Design review of the part built by this model. Coordinates are the model's own, in mm. Round coordinates to 2 decimals unless told otherwise and drop trailing zeros. Order: outer loops, then holes, each group sorted by start corner. A loop starts at its lowest first (then second) coordinate and runs counter-clockwise, first axis right, second up. Notation, with made-up numbers: (20, 38.5) - (37, 38.5) arc R20 ccw to (37, 76.5) - close; hole circle Ø6 at (60.25, 41.25). An arc over 180 degrees is marked (long way). Write item = value, one per line.
from build123d import *

# Parameters (mm, degrees)
SKETCH_1_W                    = 615
SKETCH_1_H                    = 845
EXTRUDE_1_DEPTH               = 20
SKETCH_2_W                    = 615
SKETCH_2_H                    = 30
CUT_EXTRUDE_1_DEPTH           = 13
SKETCH_3_W                    = 30
SKETCH_3_H                    = 785
CUT_EXTRUDE_2_DEPTH           = 13
HOLE_WIZARD_M4_1_D            = 4
PATTERN_LINEAR_3_COUNT        = 8
PATTERN_LINEAR_3_PITCH        = 101
PATTERN_LINEAR_4_COUNT        = 6
PATTERN_LINEAR_4_PITCH        = 97
SKETCH_15_W                   = 617
SKETCH_15_H                   = 847
SKETCH_15_W_2                 = 615
SKETCH_15_H_2                 = 845
EXTRUDE_5_DEPTH               = 7
SKETCH_17_R                   = 2.5
CUT_EXTRUDE_3_DEPTH           = 20
HOLE_WIZARD_M12_2_D           = 13.5
HOLE_WIZARD_M12_2_CBORE_D     = 19
HOLE_WIZARD_M12_2_CBORE_DEPTH = 12.5
PATTERN_LINEAR_7_COUNT        = 2
PATTERN_LINEAR_7_PITCH        = 680


with BuildPart() as part:
    # 草图1 → 拉伸1 (new body)
    with BuildSketch(Plane(origin=(0, 0, 0), x_dir=(1, 0, 0), z_dir=(0, 1, 0))):
        with Locations((307.5, 422.5)):
            Rectangle(SKETCH_1_W, SKETCH_1_H)
    extrude(amount=EXTRUDE_1_DEPTH)

    # 草图2 → 切除-拉伸1 (cut)
    with BuildSketch(Plane(origin=(0, 20, 0), x_dir=(-1, 0, 0), z_dir=(0, 1, 0))):
        with Locations((-307.5, -830)):
            Rectangle(SKETCH_2_W, SKETCH_2_H)
        with Locations((-307.5, -15)):
            Rectangle(SKETCH_2_W, SKETCH_2_H)
    extrude(amount=-CUT_EXTRUDE_1_DEPTH, mode=Mode.SUBTRACT)

    # 草图3 → 切除-拉伸2 (cut)
    with BuildSketch(Plane(origin=(0, 20, 0), x_dir=(-1, 0, 0), z_dir=(0, 1, 0))):
        with Locations((-600, -422.5)):
            Rectangle(SKETCH_3_W, SKETCH_3_H)
        with Locations((-15, -422.5)):
            Rectangle(SKETCH_3_W, SKETCH_3_H)
    extrude(amount=-CUT_EXTRUDE_2_DEPTH, mode=Mode.SUBTRACT)

    # M4 螺纹孔1 (through all)
    with Locations(Plane(origin=(598.5, 7, -826.5), x_dir=(0, 0, 1), z_dir=(0, 1, 0))):
        with Locations((0, 0), (0, -582), (808, -582), (808, 0)):
            hole_wizard_m4_1 = Hole(HOLE_WIZARD_M4_1_D / 2)

    # 阵列(线性)3: M4 螺纹孔1 ×8
    with Locations(*[(0, 0, i * PATTERN_LINEAR_3_PITCH) for i in range(1, PATTERN_LINEAR_3_COUNT)]):
        add(hole_wizard_m4_1, mode=Mode.SUBTRACT)

    # 阵列(线性)4: M4 螺纹孔1 ×6
    with Locations(*[(-i * PATTERN_LINEAR_4_PITCH, 0, 0) for i in range(1, PATTERN_LINEAR_4_COUNT)]):
        add(hole_wizard_m4_1, mode=Mode.SUBTRACT)

    # 草图15 → 凸台-拉伸5 (add)
    with BuildSketch(Plane(origin=(0, 7, 0), x_dir=(1, 0, 0), z_dir=(0, 1, 0))):
        with Locations((307.5, 422.5)):
            Rectangle(SKETCH_15_W, SKETCH_15_H)
        with Locations((307.5, 422.5)):
            Rectangle(SKETCH_15_W_2, SKETCH_15_H_2, mode=Mode.SUBTRACT)
    extrude(amount=-EXTRUDE_5_DEPTH)

    # 草图17 → 切除-拉伸3 (cut)
    with BuildSketch(Plane(origin=(0, 20, 0), x_dir=(1, 0, 0), z_dir=(0, 1, 0))):
        with Locations(Location((77.5, 82.5, 0), (0, 0, 270))):
            Circle(SKETCH_17_R)
        with Locations(Location((537.5, 82.5, 0), (0, 0, 270))):
            Circle(SKETCH_17_R)
    extrude(amount=-CUT_EXTRUDE_3_DEPTH, mode=Mode.SUBTRACT)

    # M12 六角头螺栓的柱形沉头孔2 (through all)
    with Locations(Plane(origin=(0, 20, 0), x_dir=(-1, 0, 0), z_dir=(0, 1, 0))):
        with Locations((-77.5, -82.5), (-537.5, -82.5)):
            hole_wizard_m12_2 = CounterBoreHole(HOLE_WIZARD_M12_2_D / 2, HOLE_WIZARD_M12_2_CBORE_D / 2, HOLE_WIZARD_M12_2_CBORE_DEPTH)

    # 阵列(线性)7: M12 六角头螺栓的柱形沉头孔2 ×2
    with Locations(*[(0, 0, -i * PATTERN_LINEAR_7_PITCH) for i in range(1, PATTERN_LINEAR_7_COUNT)]):
        add(hole_wizard_m12_2, mode=Mode.SUBTRACT)


solid = part.part
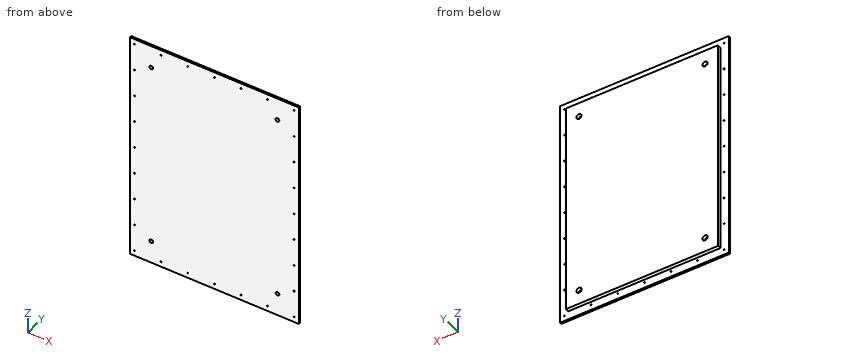
1) To check wall thickness, follow L1, parallel to Z at x = 404.5, y = 5.25; L2, parallel to X at y = 5.75, z = -762.5; L3, parallel to X at y = 17.5, z = -762.5. State the ranges of each line that lie inside material, in increasing order. Write a range as from..to.
Findings:
L1 = -846..-828.5, -824.5..-20.5, -16.5..1
L2 = -1..70.75, 84.25..530.75, 544.25..616
L3 = 30..68, 87..528, 547..585
2) Clearance check with flat-ended pins moving along their axes: pin 1 Ø10.5 at (y, z) = (16.5, -566.5) entering from +X; pin 2 Ø4.5 at (x, z) = (16.5, -321.5) entering from +Y; pin 3 Ø1 at (x, y) = (309, 13) entering from +Z. State where each tip first meets the part, or that it passes through.
Findings:
pin_1 = 585
pin_2 = 7
pin_3 = -30
3) We need section A-A on y = 12.5. Write out the cut boundary in (x, z), and give its area (3 significant figures).
Findings:
outline = (30, -815) - (585, -815) - (585, -30) - (30, -30) - close; hole circle Ø19 at (77.5, -762.5); hole circle Ø19 at (77.5, -82.5); hole circle Ø19 at (537.5, -762.5); hole circle Ø19 at (537.5, -82.5)
area = 435,000 mm^2
4) We need section B-B on z = -456. Write out the cut boundary in (x, y).
Findings:
outline = (-1, 0) - (616, 0) - (616, 7) - (585, 7) - (585, 20) - (30, 20) - (30, 7) - (-1, 7) - close
5) We need section C-C on x = 360. Write out the cut boundary in (y, z).
Findings:
outline = (0, -846) - (7, -846) - (7, -815) - (20, -815) - (20, -30) - (7, -30) - (7, 1) - (0, 1) - close
